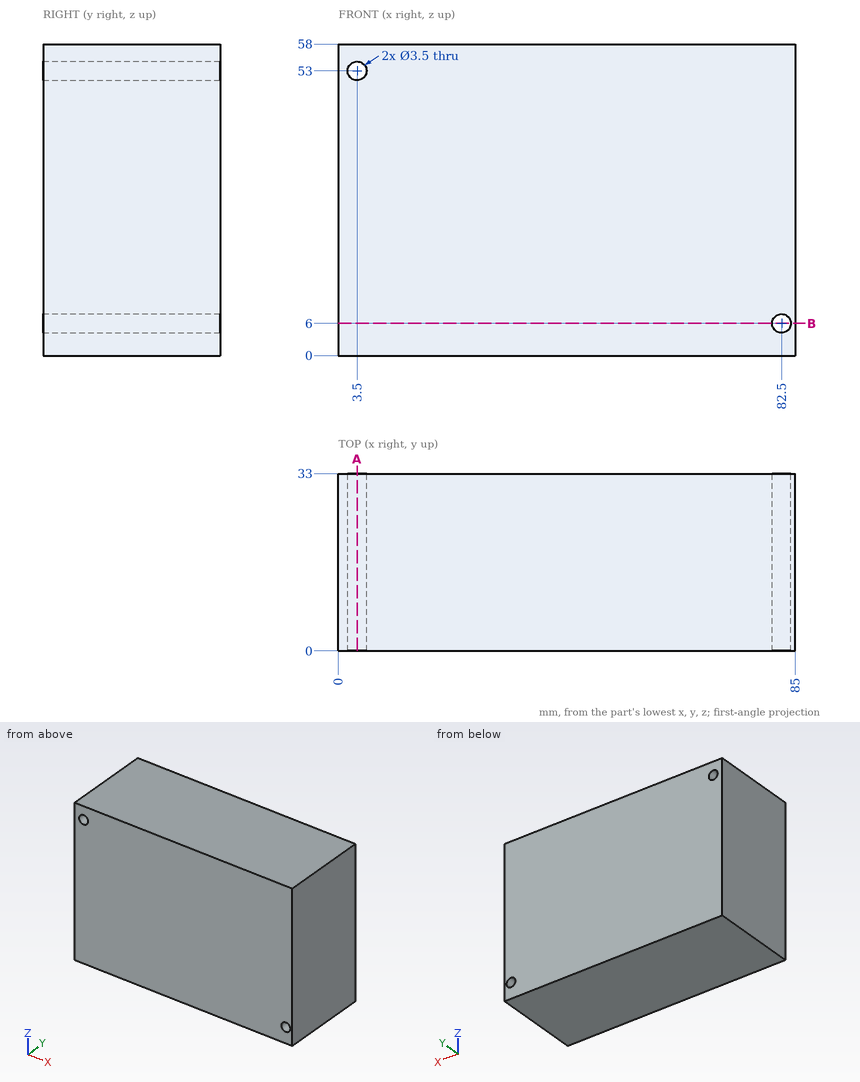
Can you work these out from the drawing? Everything is in mm from the part's minimum corner. Coordinates: 2 decimals unless noted, no trailing zeros. Write each loop counter-clockwise with the first axis right and the second up, starting at its lowest first coordinate (ties: lowest second). Pieces come first, ordered by that corner, then holes. Notation, with made-up numbers: (-2.75, 23) -> (22.25, 23) arc R25 ccw to (22.25, 60) -> close; hole circle Ø2 at (75, 73). An arc over 180 degrees is marked (long way). Write item = value, one per line.
(1) For pin 1 (3 mm diameter, centred on x = 3.5, z = 53, fed in from -Y), with a flat end and sliding along its axis, tell me the tip position at first contact or that it passes through.
Verdict:
pin_1 = through
(2) Imagine slicing it at A-A (x = 3.5). Please give me the cut outline in (y, z).
Verdict:
outline = (0, 0) -> (33, 0) -> (33, 51.25) -> (0, 51.25) -> close; (0, 54.75) -> (33, 54.75) -> (33, 58) -> (0, 58) -> close
(3) If I drill on probe 1 along Z at (x, y) = (3.5, 21.5); probe 2 along X at (y, z) = (15, 6); probe 3 along X at (y, z) = (11.5, 53), over which ranges is the centre line in solid material (lowest first)?
Verdict:
probe_1 = 0 to 51.25, 54.75 to 58
probe_2 = 0 to 80.75, 84.25 to 85
probe_3 = 0 to 1.75, 5.25 to 85
(4) Imagine slicing it at B-B (z = 6). Please give me the cut outline in (x, y), and give its area (3 significant figures).
Verdict:
outline = (0, 0) -> (80.75, 0) -> (80.75, 33) -> (0, 33) -> close; (84.25, 0) -> (85, 0) -> (85, 33) -> (84.25, 33) -> close
area = 2,690 mm^2
